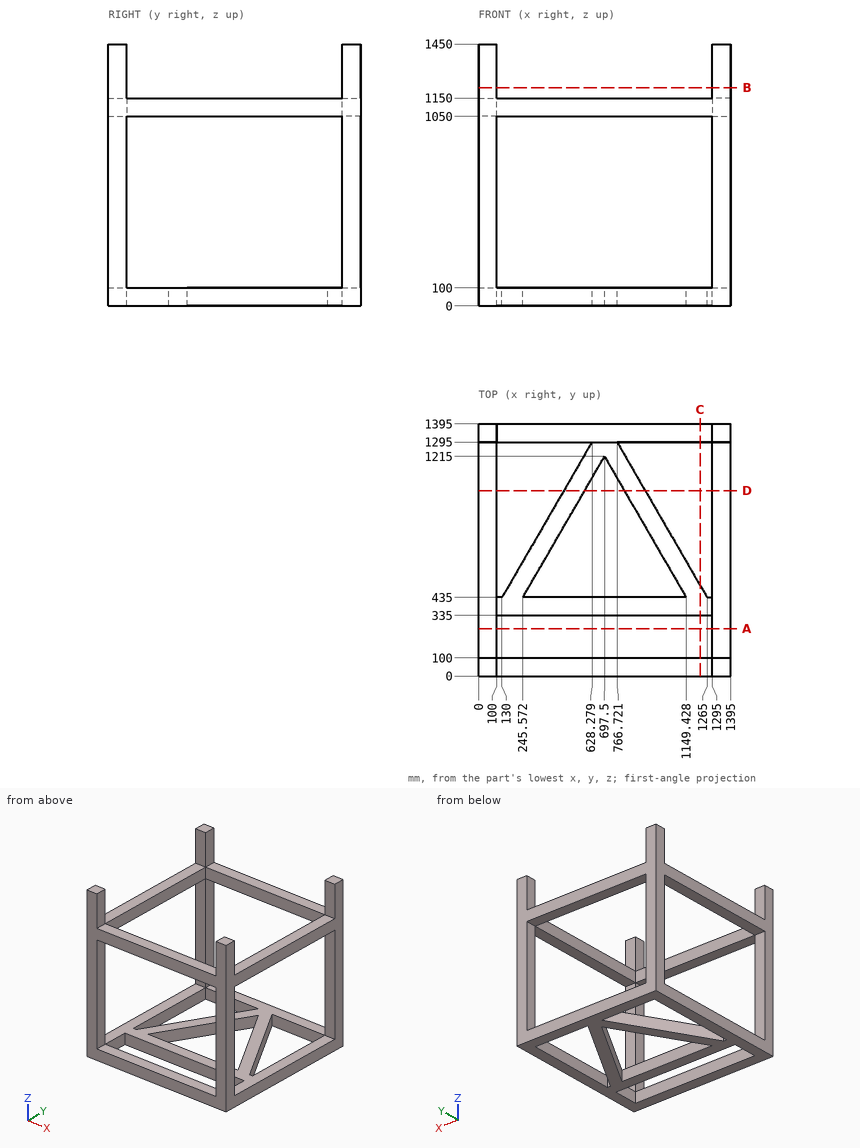
Geometry check sheet. Reference: drawing and pictorial views, mm from the part's lowest x, y, z. Coordinates: 2 decimals unless noted, no trailing zeros. Loops run counter-clockwise (first coordinate to the right, second up) from the corner with the lowest first, then second, coordinate; pieces in that order, holes last.
1) Sectioned sample at B-B (z = 1208). Record the boundary of the cut face in (x, y), and give its area (3 significant figures).
2) Material ranges on probe 1 along X at (y, z) = (1301.5, 916.5); probe 2 along Z at (x, y) = (65, 1060); probe 3 along Z at (x, y) = (668, 1208.5), recorded low to high.
3) Gauge pin test, flat end, axial feed: pin 1 (2 mm diameter, centred on x = 227, y = 513.5, fed in from +Z). Record the tip position at first contact, or that the pin passes through.
4) Sectioned sample at A-A (y = 262). Record the boundary of the cut face in (x, z).
5) Sectioned sample at C-C (x = 1227). Record the boundary of the cut face in (y, z) (1 decimal).
6) Sectioned sample at D-D (y = 1025.5). Record the boundary of the cut face in (x, z) (1 decimal), and give its area (3 significant figures).
Check sheet entries:
1. outline: (0, 0) - (100, 0) - (100, 100) - (0, 100) - close; (0, 1295) - (100, 1295) - (100, 1395) - (0, 1395) - close; (1295, 0) - (1395, 0) - (1395, 100) - (1295, 100) - close; (1295, 1295) - (1395, 1295) - (1395, 1395) - (1295, 1395) - close
1. area: 40,000 mm2
2. probe 1: x = 0 to 100, 1295 to 1395
2. probe 2: z = 0 to 100, 1050 to 1150
2. probe 3: z = 0 to 100
3. pin 1: stops at z = 100
4. outline: (0, 0) - (100, 0) - (100, 100) - (0, 100) - close; (0, 1050) - (100, 1050) - (100, 1150) - (0, 1150) - close; (1295, 0) - (1395, 0) - (1395, 100) - (1295, 100) - close; (1295, 1050) - (1395, 1050) - (1395, 1150) - (1295, 1150) - close
5. outline: (0, 0) - (100, 0) - (100, 100) - (0, 100) - close; (0, 1050) - (100, 1050) - (100, 1150) - (0, 1150) - close; (335, 0) - (500.6, 0) - (500.6, 100) - (335, 100) - close; (1295, 0) - (1395, 0) - (1395, 100) - (1295, 100) - close; (1295, 1050) - (1395, 1050) - (1395, 1150) - (1295, 1150) - close
6. outline: (0, 0) - (100, 0) - (100, 100) - (0, 100) - close; (0, 1050) - (100, 1050) - (100, 1150) - (0, 1150) - close; (472.1, 0) - (587.7, 0) - (587.7, 100) - (472.1, 100) - close; (807.3, 0) - (922.9, 0) - (922.9, 100) - (807.3, 100) - close; (1295, 0) - (1395, 0) - (1395, 100) - (1295, 100) - close; (1295, 1050) - (1395, 1050) - (1395, 1150) - (1295, 1150) - close
6. area: 63,100 mm2
